from build123d import *

# Parameters (mm, degrees)
SKETCH1_R           = 12
BOSS_EXTRUDE1_DEPTH = 5
SKETCH2_R           = 18
BOSS_EXTRUDE2_DEPTH = 5


with BuildPart() as part:
    # Sketch1 → Boss-Extrude1 (new body)
    with BuildSketch(Plane.XY):
        Circle(SKETCH1_R)
    extrude(amount=BOSS_EXTRUDE1_DEPTH)

    # Sketch2 → Boss-Extrude2 (add)
    with BuildSketch(Plane.XY.offset(5)):
        Circle(SKETCH2_R)
    extrude(amount=BOSS_EXTRUDE2_DEPTH)

    # Sketch3 → Revolve1 (revolve)
    with BuildSketch(Plane(origin=(0, 0, 0), x_dir=(0, 0, -1), z_dir=(1, 0, 0)), mode=Mode.PRIVATE) as revolve1_sk:
        Polygon((-10, 0), (-10, 12), (-40.959117986, 10.065055126), (-48, 6), (-48, 0), align=None)
    revolve(revolve1_sk.sketch.rotate(Axis((0, 0, 48), (0, 0, -1)), 90), axis=Axis((0, 0, 48), (0, 0, -1)))

    # Sketch5 → Cut-Revolve1 (revolve, cut)
    with BuildSketch(Plane(origin=(0, 0, 0), x_dir=(1, 0, 0), z_dir=(0, 1, 0)), mode=Mode.PRIVATE) as cut_revolve1_sk:
        Polygon((0, -48), (5, -48), (8, 0), (0, 0), align=None)
    revolve(cut_revolve1_sk.sketch.rotate(Axis((0, 0, 0), (0, 0, 1)), 180), axis=Axis((0, 0, 0), (0, 0, 1)), mode=Mode.SUBTRACT)


solid = part.part
CAD build for the part. Positions are in the model's coordinates, mm. A direction names the side the tool comes from. Coordinates: 2 decimals unless noted, no trailing zeros. Write each loop counter-clockwise with the first axis right and the second up, starting at its lowest first coordinate (ties: lowest second). Pieces come first, ordered by that corner, then holes. Notation, with made-up numbers: (75.5, -35) - (108.5, -35) arc R14 ccw to (108.5, -8) - close; hole circle Ø4 at (66.25, 18.25). An arc over 180 degrees is marked (long way). Use a Markdown table: item, result. Add a question column.
Item 1: Band-saw the part on A-A, the plane x = 0. Give the cut face in (y, z), and give its area (3 significant figures).
Item 2: Band-saw the part on D-D, the plane x = -14. Give the cut face in (y, z).
Item 3: 3-axis set-ups, long thin cutter, end or side, ignore diameter. For faces 1 (the face through (-2.343, 17.847, 7.465)), 2 (the face through (-11.99, 0.53, 2.46)), 3 (the face through (4, -12, 10)): which of +Z, -Z, +X, -X, +Y, -Y reach the whole face in a straight line?
Item 4: Drill centre lines: L1, parallel to Z at x = 1.5, y = -14; L2, parallel to Y at x = -1.5, z = 17; L3, parallel to X at y = 2, z = 31.5. Where is each one in solid material? Low to high. Write a range as from..to.
Item 5: Band-saw the part on C-C, the plane z = 33. Give the cut face in (x, y) (1 decimal), and give its area (3 significant figures).
Item 6: Mould opens along Y. For faces 4 (the face through (-4, -4, 48)), 5 (the face through (-6.22, -1.96, 23.66)), 6 (the face through (10.51, -3.31, 25.7)) say: pulls with the +Y half, pulls with the -Y half, needs draft (parallel to the pull), parting line crosses it, or undercut.
Item 7: Flat gauge pins, fed straight in: pin 1 (5 mm diameter, centred on y = 11, z = 27, fed in from -X); pin 2 (8 mm diameter, centred on y = 10.5, z = 6, fed in from -X); pin 3 (1 mm diameter, centred on y = 11, z = 9.5, fed in from -X). Where does each tip first touch, or does it go through?
Numbers:
| question | item | result |
|---|---|---|
| 1 | outline | (-18, 5) - (-12, 5) - (-12, 0) - (-8, 0) - (-5, 48) - (-6, 48) - (-10.07, 40.96) - (-12, 10) - (-18, 10) - close; (5, 48) - (8, 0) - (12, 0) - (12, 5) - (18, 5) - (18, 10) - (12, 10) - (10.07, 40.96) - (6, 48) - close |
| 1 | area | 472 mm2 |
| 2 | outline | (-11.31, 5) - (11.31, 5) - (11.31, 10) - (-11.31, 10) - close |
| 3 | face 1 | +Z, -Z |
| 3 | face 2 | -Z |
| 3 | face 3 | +Z |
| 4 | L1 | 5..10 |
| 4 | L2 | -11.46..-6.77, 6.77..11.46 |
| 4 | L3 | -10.47..-5.69, 5.69..10.47 |
| 5 | outline | circle Ø21.1 at (0, 0); hole circle Ø11.9 at (0, 0) |
| 5 | area | 240 mm2 |
| 6 | face 4 | needs draft |
| 6 | face 5 | undercut |
| 6 | face 6 | parting line crosses it |
| 7 | pin 1 | x = -6.89 |
| 7 | pin 2 | x = -16.79 |
| 7 | pin 3 | x = -14.62 |
